Build history of the part. All positions in model axes, mm. A direction names the side the tool comes from. Give positions to 0.01 mm unless a question says otherwise; leave off trailing zeros. Write each loop counter-clockwise with the first axis right and the second up, starting at its lowest first coordinate (ties: lowest second). Pieces come first, ordered by that corner, then holes. Notation, with made-up numbers: M 80.25,75 L 119.25,75 A20 ccw 119.25,82 Z; hole C 6.25,-34.5 d7. An arc over 180 degrees is marked long. Return JSON: item names as keys, results as strings. Group by question number.
Q1. Band-saw the part on D-D, the plane y = 10. Give the cut face in (x, z).
Q2. Band-saw the part on B-B, the plane z = -2. Give the cut face in (x, y).
Q3. Wall check: probe 1 along Y at (x, z) = (-0.5, 6.75); probe 2 along Y at (x, z) = (3, -2); probe 3 along Z at (x, y) = (-0.75, 1). Give the ranges that are in metal, low to high.
Q4. Band-saw the part on A-A, the plane y = 28.5. Give the cut face in (x, z), then the cut area to 3 significant figures.
Q5. Flat gauge pins, fed straight in: pin 1 Ø2 at (x, y) = (1.5, 4.5) entering from +Z; pin 2 Ø1.5 at (y, z) = (27, -2.5) entering from +X. Where does each tip first touch, or does it go through?
Q6. Band-saw the part on C-C, the plane x = 2.25. Give the cut face in (y, z), then the cut area to 3 significant figures.
Q7. Tool access for faces 4 (the flat face through (1.213, 28.535, -4.582)), 5 (the flat face through (-5.2, 31, -0.1)): list every direction of +Z, -Z, +X, -X, +Y, -Y with a clear straight run to the whole face (end or side of a thin tool).
Q8. Pull direction X, two halves, no side cores. Call faces 1 (the cylindrical face through (-4.88, 12.32, -1.08)), 2 (the flat face through (0, 26, 0)), 3 (the flat face through (-5.2, 25, -0.1)): +X half, -X half, draft (parallel to the pull), parting line (faces both ways), or undercut.
from build123d import *

# Parameters (mm, degrees)
SKETCH1_R           = 5
BOSS_EXTRUDE1_DEPTH = 25
SKETCH2_R           = 8
BOSS_EXTRUDE2_DEPTH = 6
CUT_EXTRUDE1_DEPTH  = 5


with BuildPart() as part:
    # Sketch1 → Boss-Extrude1 (new body)
    with BuildSketch(Plane(origin=(0, 0, 0), x_dir=(1, 0, 0), z_dir=(0, 1, 0))):
        with Locations(Location((0, 0, 0), (0, 0, 270))):
            Circle(SKETCH1_R)
    extrude(amount=BOSS_EXTRUDE1_DEPTH)

    # Sketch2 → Boss-Extrude2 (add)
    with BuildSketch(Plane(origin=(0, 25, 0), x_dir=(1, 0, 0), z_dir=(0, 1, 0))):
        with Locations(Location((0, 0, 0), (0, 0, 270))):
            Circle(SKETCH2_R)
    extrude(amount=BOSS_EXTRUDE2_DEPTH)

    # Sketch3 → Cut-Extrude1 (cut)
    with BuildSketch(Plane(origin=(0, 31, 0), x_dir=(1, 0, 0), z_dir=(0, 1, 0))):
        Polygon((-1.474961989, 5.269810816), (-5.301271034, 1.357550856), (-3.826309045, -3.91225996), (1.474961989, -5.269810816), (5.301271034, -1.357550856), (3.826309045, 3.91225996), align=None)
    extrude(amount=-CUT_EXTRUDE1_DEPTH, mode=Mode.SUBTRACT)


solid = part.part
From the geometry:
{
 "1": {"outline": "C 0,0 d10"},
 "2": {"outline": "M -7.75,25 L -4.58,25 L -4.58,0 L 4.58,0 L 4.58,25 L 7.75,25 L 7.75,31 L 4.36,31 L 4.36,26 L -4.67,26 L -4.67,31 L -7.75,31 Z"},
 "3": {"probe 1": "y = 25 to 31", "probe 2": "y = 0 to 26", "probe 3": "z = -4.94 to 4.94"},
 "4": {"outline": "C 0,0 d16; hole M -5.3,-1.36 L -1.47,-5.27 L 3.83,-3.91 L 5.3,1.36 L 1.47,5.27 L -3.83,3.91 Z", "area": "123 mm^2"},
 "5": {"pin 1": "stops at z = 4.97", "pin 2": "stops at x = 7.81"},
 "6": {"outline": "M 0,-4.47 L 25,-4.47 L 25,-7.68 L 31,-7.68 L 31,-4.32 L 26,-4.32 L 26,4.48 L 31,4.48 L 31,7.68 L 25,7.68 L 25,4.47 L 0,4.47 Z", "area": "271 mm^2"},
 "7": {"face 4": "+Y", "face 5": "+Z, -Z, +X, -X, +Y"},
 "8": {"face 1": "parting line", "face 2": "undercut", "face 3": "draft"}
}
